from build123d import *

# Parameters (mm, degrees)
BRACKET_L_BODY_DEPTH    = 20
LIP_FLANGE_DEPTH        = 1.25
END_PLATE_DEPTH         = 1.25
GUSSET_A_28_75X40_DEPTH = 1.25
GUSSET_B_27_5X40_DEPTH  = 1.25
TAB_AND_HOLES_SKETCH_W  = 7.5
TAB_AND_HOLES_SKETCH_H  = 22.5
TAB_AND_HOLES_SKETCH_R  = 1.25
MOUNTING_TAB_DEPTH      = 3.75
MOUNTING_START          = -3.75
SKETCH8_2_R             = 1.25
MOUNTING_HOLES_DEPTH    = 3.75


with BuildPart() as part:
    # L-Profile Sketch → Bracket L-Body (new body)
    with BuildSketch(Plane.XY):
        Polygon((0, 42.5), (0, 0), (-31.25, 0), (-31.25, 1.25), (-1.25, 1.25), (-1.25, 42.5), align=None)
    extrude(amount=BRACKET_L_BODY_DEPTH)

    # Lip Flange Sketch → Lip Flange (add)
    with BuildSketch(Plane.XY.offset(20)):
        Polygon((-1.25, 42.5), (-5, 42.5), (-5, 5), (-31.25, 5), (-31.25, 1.25), (-1.25, 1.25), align=None)
    extrude(amount=-LIP_FLANGE_DEPTH)

    # End Plate Sketch → End Plate (add)
    with BuildSketch(Plane(origin=(0, 0, 0), x_dir=(-1, 0, 0), z_dir=(0, 0, -1))):
        Polygon((0, 42.5), (1.25, 42.5), (5, 42.5), (5, 5), (31.25, 5), (31.25, 1.25), (31.25, 0), (0, 0), align=None)
    extrude(amount=-END_PLATE_DEPTH)

    # Gusset A Sketch → Gusset A 28.75x40 (add)
    with BuildSketch(Plane.XY.offset(1.25)):
        Polygon((-28.75, 1.25), (-1.25, 41.25), (-1.25, 1.25), align=None)
    extrude(amount=GUSSET_A_28_75X40_DEPTH)

    # Gusset B Sketch → Gusset B 27.5x40 (add)
    with BuildSketch(Plane(origin=(0, 0, 18.75), x_dir=(-1, 0, 0), z_dir=(0, 0, -1))):
        Polygon((1.25, 41.25), (28.75, 1.25), (1.25, 1.25), align=None)
    extrude(amount=GUSSET_B_27_5X40_DEPTH)

    # Tab And Holes Sketch → Mounting Tab (add)
    with BuildSketch(Plane.ZY.offset(1.25)):
        with Locations((10, 28.75)):
            Rectangle(TAB_AND_HOLES_SKETCH_W, TAB_AND_HOLES_SKETCH_H)
        with Locations(Location((10, 35, 0), (0, 0, 270))):
            Circle(TAB_AND_HOLES_SKETCH_R, mode=Mode.SUBTRACT)
        with Locations(Location((10, 25, 0), (0, 0, 270))):
            Circle(TAB_AND_HOLES_SKETCH_R, mode=Mode.SUBTRACT)
    extrude(amount=MOUNTING_TAB_DEPTH)

    # Sketch8_2 → Mounting Holes (cut)
    with BuildSketch(Plane.ZY.offset(1.25).offset(MOUNTING_START)):
        with Locations(Location((10, 35, 0), (0, 0, 270))):
            Circle(SKETCH8_2_R)
        with Locations(Location((10, 25, 0), (0, 0, 270))):
            Circle(SKETCH8_2_R)
    extrude(amount=MOUNTING_HOLES_DEPTH, mode=Mode.SUBTRACT)


solid = part.part
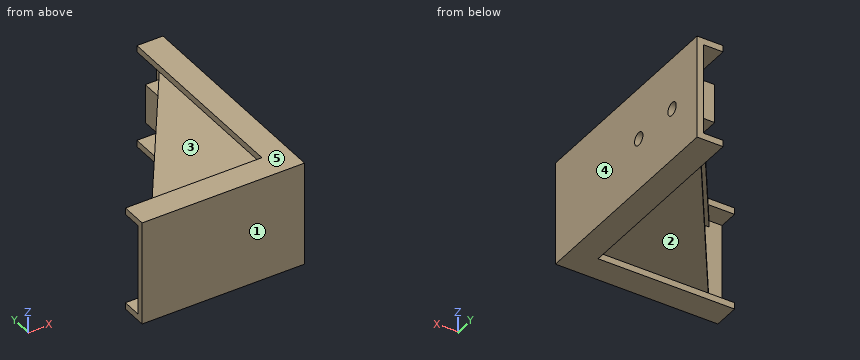
Can you work these out from the model? Positions are in its coordinate system, mm. Face numbers are marked on the shaded views. A direction names the side the tool comes from. Give positions to 0.01 mm unless a question says otherwise; leave off trailing zeros. Loops run counter-clockwise (first coordinate to the right, second up) from the corner with the lowest first, then second, coordinate; pieces in that order, holes last. Notation, with made-up numbers: (22.25, 73) - (32.25, 73) arc R10 ccw to (32.25, 79) - close; hole circle Ø5 at (-22, 75). An arc over 180 degrees is marked (long way). Answer as a JSON object with one key per item and string values.
Q1. Will these pins go through, and if not, where does the flat tip stop? P1, Ø0.6, axis at x = -18, z = 19.5, coming from the +Y side; P2, Ø6, axis at y = 26, z = 8.5, coming from the -X side; P3, Ø1, axis at x = -25, z = 11.5, coming from the +Y side.
Geometry says:
{"P1": "y = 5", "P2": "x = -5", "P3": "y = 1.25"}
Q2. If I drill on L1, parallel to Z at x = -3, y = 35; L2, parallel to Y at x = -1.8, z = 10; L3, parallel to Z at x = -5.5, y = 29, over which ranges is the centre line in solid material (lowest first)?
Geometry says:
{"L1": "0 to 2.5, 6.25 to 8.75, 11.25 to 13.75, 17.5 to 20", "L2": "0 to 1.25, 17.5 to 23.75, 26.25 to 33.75, 36.25 to 40", "L3": "1.25 to 2.5, 17.5 to 18.75"}
Q3. If we mould it in two halves opening along X, with no side actions, what happens to the marked faces 4 and 5? For each: pulls with the +X half, pulls with the -X half, needs draft (parallel to the pull), parting line crosses it, or undercut.
Geometry says:
{"face 4": "pulls with the +X half", "face 5": "needs draft"}
Q4. Imagine slicing it at A-A on z = 10. Write out the boundary of the cut face in (x, y).
Geometry says:
{"outline": "(-31.25, 0) - (0, 0) - (0, 23.75) - (-5, 23.75) - (-5, 17.5) - (-1.25, 17.5) - (-1.25, 1.25) - (-31.25, 1.25) - close; (-5, 26.25) - (0, 26.25) - (0, 33.75) - (-5, 33.75) - close; (-5, 36.25) - (0, 36.25) - (0, 42.5) - (-1.25, 42.5) - (-1.25, 40) - (-5, 40) - close"}
Q5. Imagine slicing it at B-B on y = 35. Write out the boundary of the cut face in (x, z).
Geometry says:
{"outline": "(-5.55, 1.25) - (-5, 1.25) - (-5, 0) - (0, 0) - (0, 8.75) - (-5, 8.75) - (-5, 6.25) - (-1.25, 6.25) - (-1.25, 2.5) - (-5.55, 2.5) - close; (-5.55, 17.5) - (-1.25, 17.5) - (-1.25, 13.75) - (-5, 13.75) - (-5, 11.25) - (0, 11.25) - (0, 20) - (-5, 20) - (-5, 18.75) - (-5.55, 18.75) - close"}
Q6. Imagine slicing it at C-C on x = -6. Write out the boundary of the cut face in (y, z), plus the area to 3 significant figures.
Geometry says:
{"outline": "(0, 0) - (5, 0) - (5, 1.25) - (34.34, 1.25) - (34.34, 2.5) - (1.25, 2.5) - (1.25, 17.5) - (34.34, 17.5) - (34.34, 18.75) - (5, 18.75) - (5, 20) - (0, 20) - close", "area": "117 mm²"}
Q7. Which directions (+Z, -Z, +X, -X, +Y, -Y) give clear straight access to the entire face, cutting with the end or side of a thin tool? Please do the marked faces 1, 2 and 3.
Geometry says:
{"face 1": "+Z, -Z, +X, -X, -Y", "face 2": "-Z, -X, +Y", "face 3": "+Z, -X, +Y"}
Q8. Imagine slicing it at D-D on z = 12. Write out the boundary of the cut face in (x, y).
Geometry says:
{"outline": "(-31.25, 0) - (0, 0) - (0, 42.5) - (-1.25, 42.5) - (-1.25, 40) - (-5, 40) - (-5, 17.5) - (-1.25, 17.5) - (-1.25, 1.25) - (-31.25, 1.25) - close"}
